```python
from build123d import *

# Parameters (mm, degrees)
SKETCH_1_R          = 0.7
EXTRUDE_1_DEPTH     = 2.35
SKETCH_2_R          = 4.4
EXTRUDE_2_DEPTH     = 3.5
SKETCH_3_R          = 1.425
CUT_EXTRUDE_1_DEPTH = 24.187779754
FILLET_1_R          = 0.25
SKETCH_4_R          = 4.25
SKETCH_4_R_2        = 3.5
CUT_EXTRUDE_2_DEPTH = 1
SKETCH_5_R          = 3
CUT_EXTRUDE_3_DEPTH = 1


with BuildPart() as part:
    # 草图1 → 凸台-拉伸1 (new body)
    with BuildSketch(Plane.XY):
        with BuildLine():
            Line((-4.545048295, 13.882270629), (0, 8.5))
            Line((0, 8.5), (4.591289657, 13.848716116))
            ThreePointArc((4.591289657, 13.848716116), (8.378143191, 14.486697202), (9.689930988, 10.877473971))
            Line((9.689930988, 10.877473971), (7.301272041, 4.250211371))
            Line((7.301272041, 4.250211371), (14.229040903, 2.94839595))
            ThreePointArc((14.229040903, 2.94839595), (16.674975498, -0.012124868), (14.20519039, -2.952778039))
            Line((14.20519039, -2.952778039), (7.271483148, -4.19777001))
            Line((7.271483148, -4.19777001), (9.607962353, -10.848301547))
            ThreePointArc((9.607962353, -10.848301547), (8.267043414, -14.446803451), (4.48547051, -13.778233392))
            Line((4.48547051, -13.778233392), (-0.059577785, -8.395962763))
            Line((-0.059577785, -8.395962763), (-4.650867443, -13.744678878))
            ThreePointArc((-4.650867443, -13.744678878), (-8.437720976, -14.382659965), (-9.749508773, -10.773436734))
            Line((-9.749508773, -10.773436734), (-7.360849826, -4.146174134))
            Line((-7.360849826, -4.146174134), (-14.288618688, -2.844358713))
            ThreePointArc((-14.288618688, -2.844358713), (-16.734553283, 0.116162105), (-14.264768176, 3.056815277))
            Line((-14.264768176, 3.056815277), (-7.331060933, 4.301807247))
            Line((-7.331060933, 4.301807247), (-9.667540138, 10.952338784))
            ThreePointArc((-9.667540138, 10.952338784), (-8.326621199, 14.550840688), (-4.545048295, 13.882270629))
        make_face()
        with Locations((13.675, 0)):
            Circle(SKETCH_1_R, mode=Mode.SUBTRACT)
        with Locations((10.675, 0)):
            Circle(SKETCH_1_R, mode=Mode.SUBTRACT)
        with Locations((7.675, 0)):
            Circle(SKETCH_1_R, mode=Mode.SUBTRACT)
        with Locations((3.8375, -6.646744974)):
            Circle(SKETCH_1_R, mode=Mode.SUBTRACT)
        with Locations((5.3375, -9.244821185)):
            Circle(SKETCH_1_R, mode=Mode.SUBTRACT)
        with Locations((6.8375, -11.842897397)):
            Circle(SKETCH_1_R, mode=Mode.SUBTRACT)
        with Locations((-3.8375, -6.646744974)):
            Circle(SKETCH_1_R, mode=Mode.SUBTRACT)
        with Locations((-5.3375, -9.244821185)):
            Circle(SKETCH_1_R, mode=Mode.SUBTRACT)
        with Locations((-6.8375, -11.842897397)):
            Circle(SKETCH_1_R, mode=Mode.SUBTRACT)
        with Locations((-7.675, 0)):
            Circle(SKETCH_1_R, mode=Mode.SUBTRACT)
        with Locations((-10.675, 0)):
            Circle(SKETCH_1_R, mode=Mode.SUBTRACT)
        with Locations((-13.675, 0)):
            Circle(SKETCH_1_R, mode=Mode.SUBTRACT)
        with Locations((-3.8375, 6.646744974)):
            Circle(SKETCH_1_R, mode=Mode.SUBTRACT)
        with Locations((-5.3375, 9.244821185)):
            Circle(SKETCH_1_R, mode=Mode.SUBTRACT)
        with Locations((-6.8375, 11.842897397)):
            Circle(SKETCH_1_R, mode=Mode.SUBTRACT)
        with Locations((3.8375, 6.646744974)):
            Circle(SKETCH_1_R, mode=Mode.SUBTRACT)
        with Locations((5.3375, 9.244821185)):
            Circle(SKETCH_1_R, mode=Mode.SUBTRACT)
        with Locations((6.8375, 11.842897397)):
            Circle(SKETCH_1_R, mode=Mode.SUBTRACT)
    extrude(amount=EXTRUDE_1_DEPTH)

    # 草图2 → 凸台-拉伸2 (add)
    with BuildSketch(Plane.XY.offset(2.35)):
        Circle(SKETCH_2_R)
    extrude(amount=EXTRUDE_2_DEPTH)

    # 草图3 → 切除-拉伸1 (cut, through all)
    with BuildSketch(Plane.XY.offset(5.85)):
        Circle(SKETCH_3_R)
    extrude(amount=-CUT_EXTRUDE_1_DEPTH, mode=Mode.SUBTRACT)

    # 圆角1
    fillet_1_edges = [part.edges().sort_by_distance(p)[0] for p in [
        (-4.4, 0, 5.85),
        (-1.425, 0, 5.85),
    ]]
    fillet(fillet_1_edges, radius=FILLET_1_R)

    # 草图4 → 切除-拉伸2 (cut)
    with BuildSketch(Plane(origin=(0, 0, 0), x_dir=(-1, 0, 0), z_dir=(0, 0, -1))):
        Circle(SKETCH_4_R)
        Circle(SKETCH_4_R_2, mode=Mode.SUBTRACT)
    extrude(amount=-CUT_EXTRUDE_2_DEPTH, mode=Mode.SUBTRACT)

    # 草图5 → 切除-拉伸3 (cut)
    with BuildSketch(Plane(origin=(0, 0, 0), x_dir=(-1, 0, 0), z_dir=(0, 0, -1))):
        Circle(SKETCH_5_R)
    extrude(amount=-CUT_EXTRUDE_3_DEPTH, mode=Mode.SUBTRACT)


solid = part.part
```
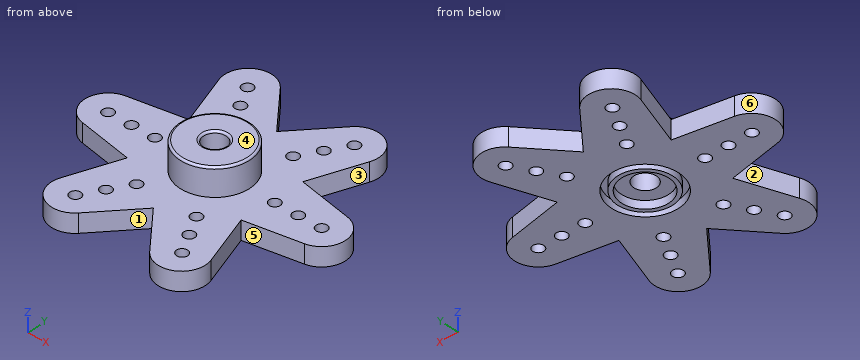
Geometry: final body of the model. Coordinates: model frame, mm. Face numbers are marked on the shaded views. A direction names the side the tool comes from. Give positions to 0.01 mm unless a question says otherwise; leave off trailing zeros. Order: outer loops, then holes, each group sorted by start corner. A loop starts at its lowest first (then second) coordinate and runs counter-clockwise, first axis right, second up. Notation, with made-up numbers: M -0.5,74.5 L 22.5,74.5 A21 cw 22.5,96.5 Z; hole C 21,47 d2. An arc over 180 degrees is marked long. Answer as CSV lines item,"result". Start each with the question number.
1) Cut plane C-C (y = 0). State how many separate pieces and enclosed holes the cut face has, then the cut area to 3 significant figures.
2) Cut plane A-A (x = -11). Output: boundary loops of the cut face in (y, z).
3) Mould query, pull axis Y, two halves, no side actions, for the marked faces 4, 5 and 6. Classes: +Y half, -Y half, draft (parallel to the pull), parting line (faces both ways), or undercut.
4) Cut plane D-D (y = 5). Output: boundary loops of the cut face in (x, z).
5) Line query: line 1 (Y direction, x = 0, z = 4.05) (3 decimals); line 2 (X direction, y = 6.5, z = 1.8); line 3 (Z direction, x = -2.5, y = -2.75). Output: solid intervals per line, ascending. Write a range as from..to.
6) Cut plane B-B (z = 3.8). Output: boundary loops of the cut face in (x, y) (3 decimals).
7) Set-up query: the marked faces 1, 2 and 3. Return all of +Z, -Z, +X, -X, +Y, -Y with unobstructed straight access to the full face (end or side cutting, diameter ignored); none if empty.
8) First-contact query: P1, Ø1.5, axis at x = 11, z = 3, coming from the +Y side; P2, Ø1.3, axis at x = 6.84, y = 11.84, coming from the -Z side; P3, Ø10, axis at x = 10, y = 8, coming from the +Z side; P4, Ø3, axis at y = 4, z = 1, coming from the +X side. Flat tips, straight axial feed; report the tip coordinate or a pass-through.
Findings below:
1,separate pieces,"8"
1,enclosed holes,"0"
1,area,"68.2 mm²"
2,outline,"M -3.46,0 L -0.62,0 L -0.62,2.35 L -3.46,2.35 Z; M 0.62,0 L 3.64,0 L 3.64,2.35 L 0.62,2.35 Z"
3,face 4,"draft"
3,face 5,"undercut"
3,face 6,"parting line"
4,outline,"M -7.58,0 L 7.57,0 L 7.57,2.35 L -7.58,2.35 Z"
5,line 1,"y = -4.4..-1.425, 1.425..4.4"
5,line 2,"x = -8.1..-4.52, -3.15..3.15, 4.52..8.11"
5,line 3,"z = 1..5.85"
6,outline,"C 0,0 d8.8; hole C 0,0 d2.85"
7,face 1,"+Z, -Z, -Y"
7,face 2,"+Z, -Z, -X"
7,face 3,"+Z, -Z, +X"
8,P1,"stops at y = 3.63"
8,P2,"passes through"
8,P3,"stops at z = 2.35"
8,P4,"stops at x = 15.33"
